Check sheet for the drawn part. Datum: minimum x, y, z corner. Units: mm. A direction names the side the tool comes from. Give positions to 0.01 mm unless a question says otherwise; leave off trailing zeros. Write each loop counter-clockwise with the first axis right and the second up, starting at its lowest first coordinate (ties: lowest second). Pieces come first, ordered by that corner, then holes.
(1) Mould release check, pull along Z, two halves, no side actions. Record for the marked faces 4, 5 and 6: +Z half, -Z half, draft (parallel to the pull), parting line (faces both ways), or undercut.
(2) Cross-section at B-B (y = 55). Record the boundary of the cut face in (x, z), and give its area (3 significant figures).
(3) Thickness scan on line 1 along Y through (x, z) = (12, 5.5); line 2 along Y through (x, z) = (35, 5.5); line 3 along X through (y, z) = (9, 6). Record the ranges inside material, lowest first.
(4) Cross-section at C-C (z = 4). Record the boundary of the cut face in (x, y).
(5) Tool access check on the marked faces 1, 2 and 3. Record the directions out of +Z, -Z, +X, -X, +Y, -Y that give a thin tool (end or side, any length) a straight path to the whole face; none if there is none.
(6) Cross-section at A-A (x = 35). Record the boundary of the cut face in (y, z).
(7) Cross-section at D-D (y = 10). Record the boundary of the cut face in (x, z).
(8) Depth check by flat-ended pin: P1, Ø3.5, axis at x = 37, y = 12, coming from the +Z side; P2, Ø7.5, axis at x = 35, y = 55, coming from the -Z side. Enter the tip coordinate at first touch or a pass-through.
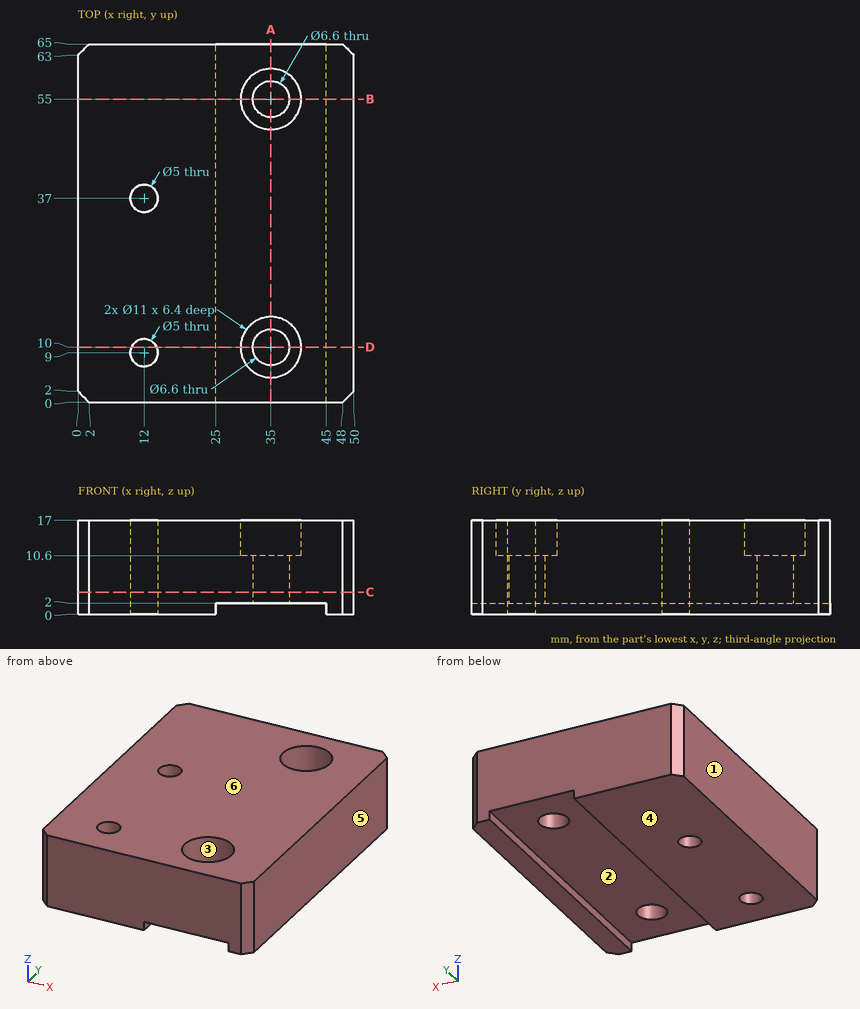
Reply:
1. face 4: -Z half
1. face 5: draft
1. face 6: +Z half
2. outline: (0, 0) - (25, 0) - (25, 2) - (31.7, 2) - (31.7, 10.6) - (29.5, 10.6) - (29.5, 17) - (0, 17) - close; (38.3, 2) - (45, 2) - (45, 0) - (50, 0) - (50, 17) - (40.5, 17) - (40.5, 10.6) - (38.3, 10.6) - close
2. area: 683 mm2
3. line 1: y = 0 to 6.5, 11.5 to 34.5, 39.5 to 65
3. line 2: y = 0 to 6.7, 13.3 to 51.7, 58.3 to 65
3. line 3: x = 0 to 9.5, 14.5 to 31.86, 38.14 to 50
4. outline: (0, 2) - (2, 0) - (48, 0) - (50, 2) - (50, 63) - (48, 65) - (2, 65) - (0, 63) - close; hole circle Ø5 at (12, 9); hole circle Ø5 at (12, 37); hole circle Ø6.6 at (35, 10); hole circle Ø6.6 at (35, 55)
5. face 1: +Z, -Z, -X, +Y, -Y
5. face 2: -Z, +Y, -Y
5. face 3: +Z
6. outline: (0, 2) - (6.7, 2) - (6.7, 10.6) - (4.5, 10.6) - (4.5, 17) - (0, 17) - close; (13.3, 2) - (51.7, 2) - (51.7, 10.6) - (49.5, 10.6) - (49.5, 17) - (15.5, 17) - (15.5, 10.6) - (13.3, 10.6) - close; (58.3, 2) - (65, 2) - (65, 17) - (60.5, 17) - (60.5, 10.6) - (58.3, 10.6) - close
7. outline: (0, 0) - (9.71, 0) - (9.71, 17) - (0, 17) - close; (14.29, 0) - (25, 0) - (25, 2) - (31.7, 2) - (31.7, 10.6) - (29.5, 10.6) - (29.5, 17) - (14.29, 17) - close; (38.3, 2) - (45, 2) - (45, 0) - (50, 0) - (50, 17) - (40.5, 17) - (40.5, 10.6) - (38.3, 10.6) - close
8. P1: stops at z = 10.6
8. P2: stops at z = 2
